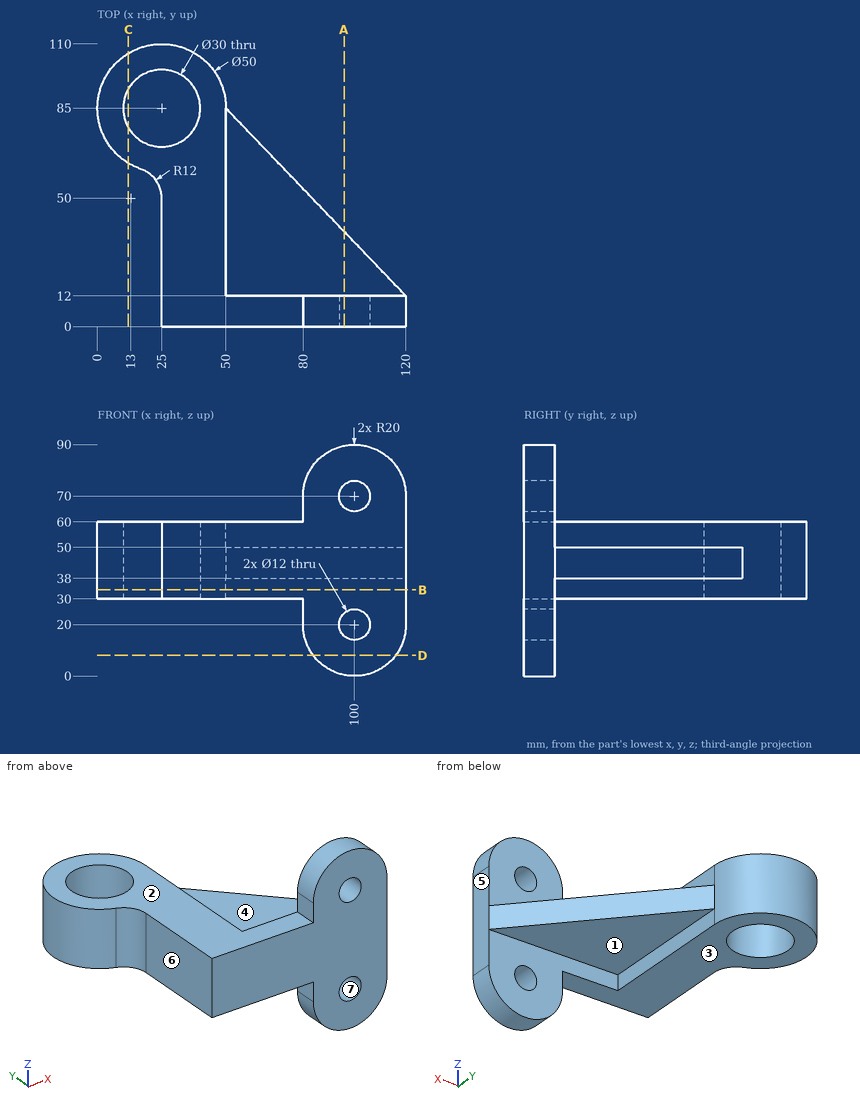
Geometry check sheet. Reference: drawing and pictorial views, mm from the part's lowest x, y, z. A direction names the side the tool comes from. Give positions to 0.01 mm unless a question says otherwise; leave off trailing zeros. Order: outer loops, then holes, each group sorted by start corner. A loop starts at its lowest first (then second) coordinate and runs counter-clockwise, first axis right, second up. Notation, with made-up numbers: M -24.5,24.25 L 21.5,24.25 A21 ccw 21.5,51.25 Z; hole C 23,25 d2. An arc over 180 degrees is marked long. Answer in a Markdown table with one row per item. Add a question column.
Q1. Access from +Z, -Z, +X, -X, +Y, -Y to the whole of each face (thin tool, end or side, straight path). Record for the marked faces 1, 2, 3 and 4.
Q2. Sectioned sample at A-A, the plane x = 96. Record the boundary of the cut face in (y, z).
Q3. Gauge pin test, flat ends, axial feed: pin 1 Ø9.5 at (x, z) = (100, 20) entering from -Y; pin 2 Ø3 at (x, z) = (38, 59.5) entering from +Y; pin 3 Ø3 at (y, z) = (59, 55) entering from +X; pin 4 Ø3 at (y, z) = (8, 23) entering from -X. Record the tip position at first contact, or that the pin passes through.
Q4. Sectioned sample at C-C, the plane x = 12. Record the boundary of the cut face in (y, z).
Q5. Release check for a two-part mould opening along X. For the marked faces 5, 6 and 7 record: released by +X, released by -X, zero draft, split by the parting line, or undercut.
Q6. Thickness scan on L1, parallel to X at y = 7.5, z = 70; L2, parallel to X at y = 11, z = 42.5; L3, parallel to Y at x = 108, z = 52.5. Record the ranges inside material, lowest first.
Q7. Sectioned sample at D-D, the plane z = 8. Record the boundary of the cut face in (x, y), and give its area (3 significant figures).
Q8. Sectioned sample at B-B, the plane z = 33.5. Record the boundary of the cut face in (x, y).
Verdict:
| question | item | result |
|---|---|---|
| 1 | face 1 | -Z, +X, +Y |
| 1 | face 2 | +Z, -X, +Y, -Y |
| 1 | face 3 | -Z, -X, +Y, -Y |
| 1 | face 4 | +Z, +X, +Y |
| 2 | outline | M 0,0.4 L 12,0.4 L 12,15.53 L 0,15.53 Z; M 0,24.47 L 12,24.47 L 12,38 L 37.03,38 L 37.03,50 L 12,50 L 12,65.53 L 0,65.53 Z; M 0,74.47 L 12,74.47 L 12,89.6 L 0,89.6 Z |
| 3 | pin 1 | through |
| 3 | pin 2 | y = 107.2 |
| 3 | pin 3 | x = 50 |
| 3 | pin 4 | x = 80 |
| 4 | outline | M 63.65,30 L 77.52,30 L 77.52,60 L 63.65,60 Z; M 92.48,30 L 106.35,30 L 106.35,60 L 92.48,60 Z |
| 5 | face 5 | released by +X |
| 5 | face 6 | released by -X |
| 5 | face 7 | undercut |
| 6 | L1 | 80 to 94, 106 to 120 |
| 6 | L2 | 25 to 120 |
| 6 | L3 | 0 to 12 |
| 7 | outline | M 84,0 L 116,0 L 116,12 L 84,12 Z |
| 7 | area | 384 mm² |
| 8 | outline | M 16.89,61.35 A12 cw 25,50 L 25,0 L 120,0 L 120,12 L 50,12 L 50,85 A25 ccw long Z; hole C 25,85 d30 |
